Check sheet for the drawn part. Datum: minimum x, y, z corner. Units: mm. Give positions to 0.01 mm unless a question says otherwise; leave off trailing zeros. Order: outer loops, then holes, each group sorted by start corner. A loop starts at its lowest first (then second) coordinate and runs counter-clockwise, first axis right, second up. Notation, with made-up numbers: M 7.25,75 L 43.25,75 A22 cw 43.25,102 Z; hole C 38,82.5 d6. An arc over 180 degrees is marked long. Answer in a Markdown table with one row per item. Add a question column.
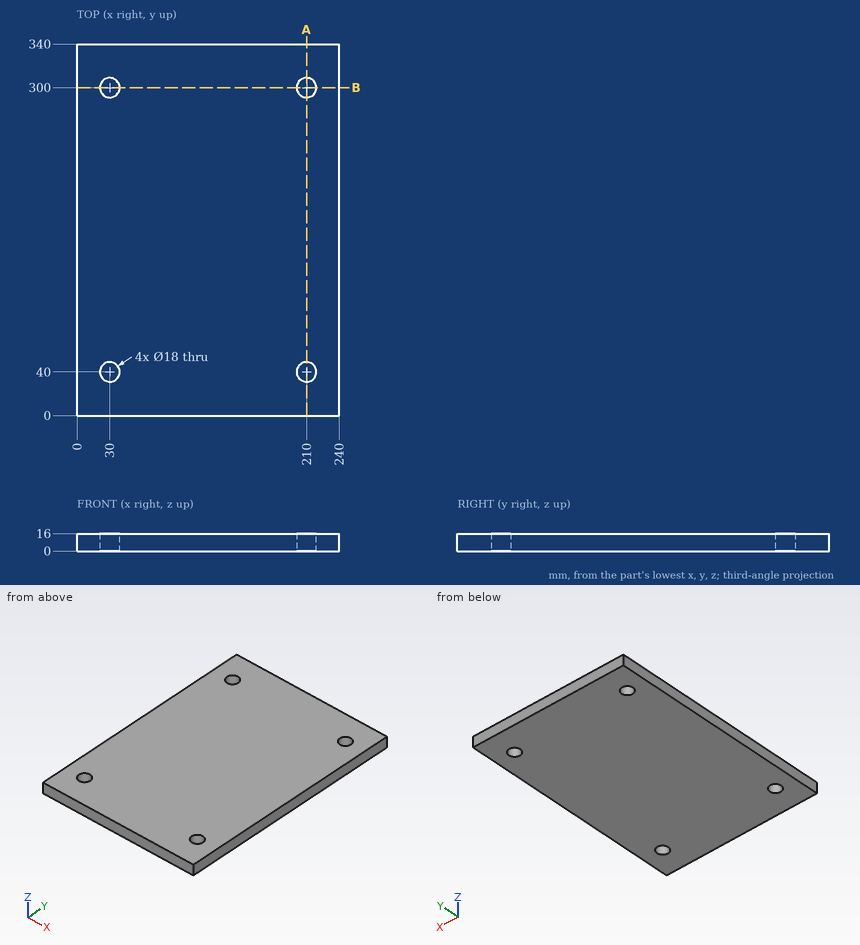
Q1. Thickness scan on probe 1 along X at (y, z) = (300, 9.75); probe 2 along Y at (x, z) = (30, 3.75); probe 3 along X at (y, z) = (295.5, 4.25). Record the ranges inside material, lowest first.
Q2. Go/stop test with a flat-tipped pin: pin 1 (14.5 mm diameter, centred on x = 210, y = 300, fed in from -Z). Record where the tip stops, or that it passes through.
Q3. Cross-section at A-A (x = 210). Record the boundary of the cut face in (y, z).
Q4. Cross-section at B-B (y = 300). Record the boundary of the cut face in (x, z).
Values follow:
| question | item | result |
|---|---|---|
| 1 | probe 1 | 0 to 21, 39 to 201, 219 to 240 |
| 1 | probe 2 | 0 to 31, 49 to 291, 309 to 340 |
| 1 | probe 3 | 0 to 22.21, 37.79 to 202.21, 217.79 to 240 |
| 2 | pin 1 | through |
| 3 | outline | M 0,0 L 31,0 L 31,16 L 0,16 Z; M 49,0 L 291,0 L 291,16 L 49,16 Z; M 309,0 L 340,0 L 340,16 L 309,16 Z |
| 4 | outline | M 0,0 L 21,0 L 21,16 L 0,16 Z; M 39,0 L 201,0 L 201,16 L 39,16 Z; M 219,0 L 240,0 L 240,16 L 219,16 Z |
